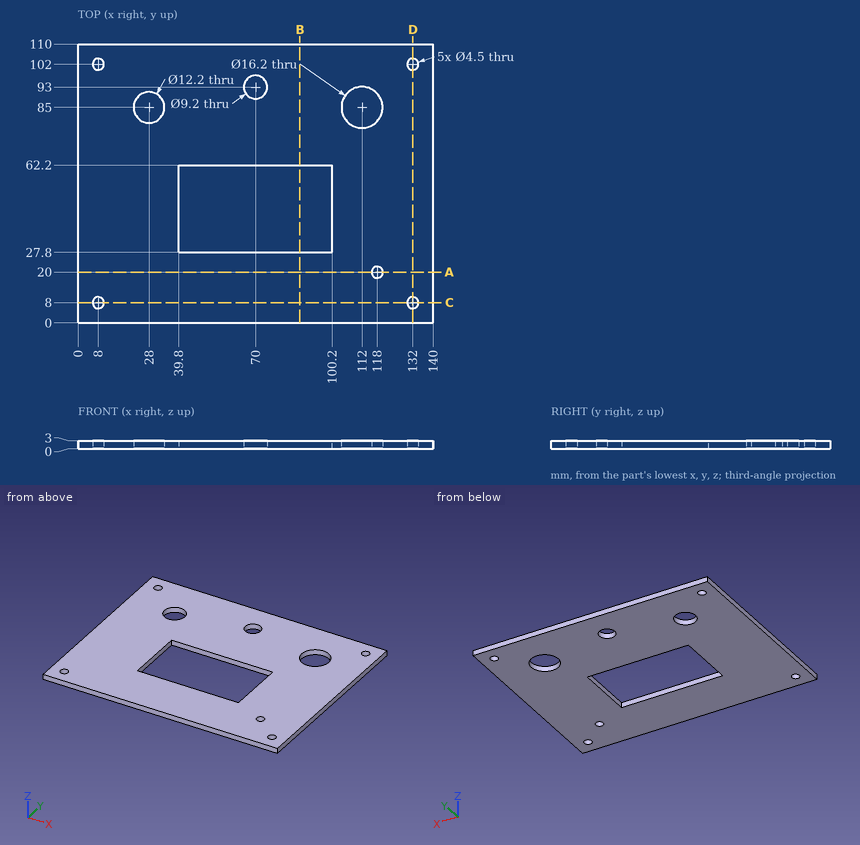
Check sheet for the drawn part. Datum: minimum x, y, z corner. Units: mm. Round coordinates to 2 decimals unless told otherwise and drop trailing zeros. Order: outer loops, then holes, each group sorted by start corner. A loop starts at its lowest first (then second) coordinate and runs counter-clockwise, first axis right, second up.
(1) Cross-section at D-D, the plane x = 132. Enter the section's corners in (y, z), and give its area (3 significant figures).
(2) Go/stop test with a flat-tipped pin: P1, Ø7, axis at x = 132, y = 8, coming from the +Z side. Record where the tip stops, or that it passes through.
(3) Scan lines: probe 1 along Y at (x, z) = (132, 2.1); probe 2 along X at (y, z) = (102, 1.1); probe 3 along Y at (x, z) = (70, 0.65). Record each from-to range of solid material in increasing order.
(4) Cross-section at A-A, the plane y = 20. Enter the section's corners in (x, z), and give its area (4 significant figures).
(5) Cross-section at B-B, the plane x = 87.5. Enter the section's corners in (y, z), and give its area (3 significant figures).
(6) Cross-section at C-C, the plane y = 8. Enter the section's corners in (x, z), and give its area (3 significant figures).
Check sheet entries:
1. outline: (0, 0) - (5.75, 0) - (5.75, 3) - (0, 3) - close; (10.25, 0) - (99.75, 0) - (99.75, 3) - (10.25, 3) - close; (104.25, 0) - (110, 0) - (110, 3) - (104.25, 3) - close
1. area: 303 mm2
2. P1: stops at z = 3
3. probe 1: y = 0 to 5.75, 10.25 to 99.75, 104.25 to 110
3. probe 2: x = 0 to 5.75, 10.25 to 129.75, 134.25 to 140
3. probe 3: y = 0 to 27.8, 62.2 to 88.4, 97.6 to 110
4. outline: (0, 0) - (115.75, 0) - (115.75, 3) - (0, 3) - close; (120.25, 0) - (140, 0) - (140, 3) - (120.25, 3) - close
4. area: 406.5 mm2
5. outline: (0, 0) - (27.8, 0) - (27.8, 3) - (0, 3) - close; (62.2, 0) - (110, 0) - (110, 3) - (62.2, 3) - close
5. area: 227 mm2
6. outline: (0, 0) - (5.75, 0) - (5.75, 3) - (0, 3) - close; (10.25, 0) - (129.75, 0) - (129.75, 3) - (10.25, 3) - close; (134.25, 0) - (140, 0) - (140, 3) - (134.25, 3) - close
6. area: 393 mm2
